```python
from build123d import *

# Parameters (mm, degrees)
CHAMFER_1_SIZE = 1


with BuildPart() as part:
    # 草图1 → 旋转1 (revolve)
    with BuildSketch(Plane(origin=(0, 0, 0), x_dir=(1, 0, 0), z_dir=(0, 1, 0)), mode=Mode.PRIVATE) as revolve_1_sk:
        Polygon((0, 16), (0, 45), (9, 45), (9, 39.8), (11, 39.8), (11, 40), (17.5, 40), (17.5, 45), (26.75, 45), (26.75, 40), (33.25, 40), (33.25, 45), (42.5, 45), (42.5, 40), (49, 40), (49, 39.8), (51, 39.8), (51, 45), (60, 45), (60, 32), (45, 32), (45, 10), (30, 10), (30, 16), align=None)
    revolve(revolve_1_sk.sketch.rotate(Axis((0, 0, 0), (1, 0, 0)), 180), axis=Axis((0, 0, 0), (1, 0, 0)))

    # 倒角1
    chamfer_1_edges = [part.edges().sort_by_distance(p)[0] for p in [
        (60, 0, -45),
        (51, 0, -45),
        (42.5, 0, -45),
        (33.25, 0, -45),
        (26.75, 0, -45),
        (17.5, 0, -45),
        (9, 0, -45),
        (0, 0, -45),
    ]]
    chamfer(chamfer_1_edges, length=CHAMFER_1_SIZE)


solid = part.part
```
CAD build for the part. Positions are in the model's coordinates, mm. A direction names the side the tool comes from. Round coordinates to 2 decimals unless told otherwise and drop trailing zeros. Order: outer loops, then holes, each group sorted by start corner. A loop starts at its lowest first (then second) coordinate and runs counter-clockwise, first axis right, second up.
Q1. Slice it at A-A (x = 20.5). Write the cut outline in (y, z), and give its area (3 significant figures).
Q2. Which spindle directions (+Z, -Z, +X, -X, +Y, -Y) get a long thin tool onto all of the face, cutting with end or side? Do faces 1 (the cylindrical face through (37.926, 39.923, 20.765)), 2 (the flat face through (45, -8, 7)), 3 (the flat face through (9, 23, -33)). Say none if no direction does.
Q3. Wall check: L1, parallel to X at y = 22, z = 38; L2, parallel to Y at x = 40.75, z = 0; L3, parallel to Y at x = 14.75, z = 0. Give the ranges that are in metal, low to high.
Q4. Drop flat-ended pins along their axis: pin 1 (3 mm diameter, centred on x = 36, z = -30, fed in from +Y); pin 2 (2 mm diameter, centred on x = 9, y = 30, fed in from +Z); pin 3 (12 mm diameter, centred on x = 17.5, z = -24.5, fed in from +Y); pin 4 (6 mm diameter, centred on y = -14, z = 18, fed in from -X). Give the stop position or say it passes through.
Q5. Two-plate mould, pull along X, no slides. Class faces 4 (the flat face through (33.25, 39, -10)), 5 (the cylindrical face through (4.549, 39.923, 20.765)), 6 (the flat face through (60, 32.4, 3.1)), 7 (the cylindrical face through (14.3, -1.76, -39.96)): pulls with the +X half, pulls with the -X half, needs draft (parallel to the pull), parting line crosses it, or undercut.
Results below:
1. outline: circle Ø90 at (0, 0); hole circle Ø32 at (0, 0)
1. area: 5,560 mm2
2. face 1: +X, -X
2. face 2: +X
2. face 3: none
3. L1: x = 0 to 9, 17.5 to 26.75, 33.25 to 42.5, 51 to 60
3. L2: y = -45 to -10, 10 to 45
3. L3: y = -40 to -16, 16 to 40
4. pin 1: stops at y = 34.82
4. pin 2: stops at z = 33.81
4. pin 3: stops at y = 40.98
4. pin 4: stops at x = 0
5. face 4: undercut
5. face 5: needs draft
5. face 6: pulls with the +X half
5. face 7: undercut
